Input: part model. Units: mm. Frame: model coordinates. Face numbers are marked on the shaded views. Coordinates: 2 decimals unless noted, no trailing zeros.
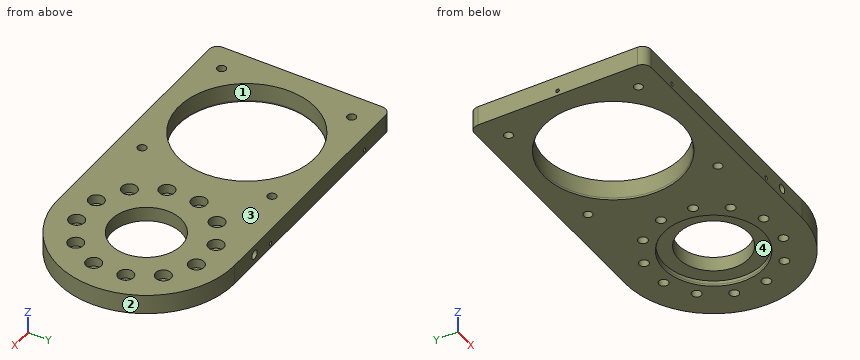
from build123d import *

# Parameters (mm, degrees)
BOSS_EXTRUDE1_DEPTH                                  = 23
FILLET1_R                                            = 10
HOLE_SIZE_PER_SOCKET_HEAD_CAP_SCREW_TYPE_D           = 11
HOLE_SIZE_PER_SOCKET_HEAD_CAP_SCREW_TYPE_CBORE_D     = 18
HOLE_SIZE_PER_SOCKET_HEAD_CAP_SCREW_TYPE_CBORE_DEPTH = 11
CIRPATTERN1_COUNT                                    = 12
SKETCH8_R                                            = 80
CUT_EXTRUDE1_DEPTH                                   = 23
SKETCH13_R                                           = 41
CUT_EXTRUDE3_DEPTH                                   = 23
SKETCH14_R                                           = 57.5
CUT_EXTRUDE4_DEPTH                                   = 6
M12_TAPPED_HOLE2_D                                   = 10.2
M5_TAPPED_HOLE1_AT_2_COUNT                           = 2
M5_TAPPED_HOLE1_AT_2_PITCH                           = 180
CHAMFER3_SIZE                                        = 2
CHAMFER3_SIZE2                                       = 0.727940469
CHAMFER4_SIZE                                        = 2
CHAMFER4_SIZE2                                       = 0.727940469
M5_TAPPED_HOLE3_D                                    = 4.2
M5_TAPPED_HOLE3_DEPTH                                = 12.4
M5_TAPPED_HOLE3_TIP                                  = 1.2618073


with BuildPart() as part:
    # Sketch1 → Boss-Extrude1 (new body)
    with BuildSketch(Plane.XY):
        with BuildLine():
            Line((0, 0), (298.3, 0))
            ThreePointArc((298.3, 0), (401.6, 103.3), (298.3, 206.6))
            Line((298.3, 206.6), (0, 206.6))
            Line((0, 206.6), (0, 0))
        make_face()
    extrude(amount=BOSS_EXTRUDE1_DEPTH)

    # Fillet1
    fillet1_edges = [part.edges().sort_by_distance(p)[0] for p in [
        (0, 206.6, 11.5),
        (0, 0, 11.5),
    ]]
    fillet(fillet1_edges, radius=FILLET1_R)

    # Hole Size per Socket Head Cap Screw Type3 (through all)
    with Locations(Plane.XY.offset(23)):
        with Locations((368.329622406, 84.53561923)):
            hole_size_per_socket_head_cap_screw_type = CounterBoreHole(HOLE_SIZE_PER_SOCKET_HEAD_CAP_SCREW_TYPE_D / 2, HOLE_SIZE_PER_SOCKET_HEAD_CAP_SCREW_TYPE_CBORE_D / 2, HOLE_SIZE_PER_SOCKET_HEAD_CAP_SCREW_TYPE_CBORE_DEPTH)

    # CirPattern1: Hole Size per Socket Head Cap Screw Type3 ×12 about axis
    cirpattern1_axis = Axis((298.3, 103.3, 0), (0, 0, 1))
    for i in range(1, CIRPATTERN1_COUNT):
        add(hole_size_per_socket_head_cap_screw_type.rotate(cirpattern1_axis, i * 360 / CIRPATTERN1_COUNT), mode=Mode.SUBTRACT)

    # Sketch8 → Cut-Extrude1 (cut)
    with BuildSketch(Plane.XY.offset(23)):
        with Locations((106.3, 103.3)):
            Circle(SKETCH8_R)
    extrude(amount=-CUT_EXTRUDE1_DEPTH, mode=Mode.SUBTRACT)

    # Sketch13 → Cut-Extrude3 (cut)
    with BuildSketch(Plane(origin=(0, 0, 0), x_dir=(-1, 0, 0), z_dir=(0, 0, -1))):
        with Locations((-298.3, 103.3)):
            Circle(SKETCH13_R)
    extrude(amount=-CUT_EXTRUDE3_DEPTH, mode=Mode.SUBTRACT)

    # Sketch14 → Cut-Extrude4 (cut)
    with BuildSketch(Plane(origin=(0, 0, 0), x_dir=(-1, 0, 0), z_dir=(0, 0, -1))):
        with Locations((-298.3, 103.3)):
            Circle(SKETCH14_R)
    extrude(amount=-CUT_EXTRUDE4_DEPTH, mode=Mode.SUBTRACT)

    # M12 Tapped Hole2 (through all)
    with Locations(Plane(origin=(0, 0, 0), x_dir=(-1, 0, 0), z_dir=(0, 0, -1))):
        with Locations((-30.286021022, 27.286021022), (-182.313978978, 27.286021022), (-30.286021022, 179.313978978), (-182.313978978, 179.313978978), (-106.3, 103.3)):
            Hole(M12_TAPPED_HOLE2_D / 2)

    # Sketch18 → M5 Tapped Hole1 (revolve, cut)
    with BuildSketch(Plane(origin=(50, 206.6, 5.5), x_dir=(0, 0, 1), z_dir=(1, 0, 0))):
        Polygon((0, 0), (0, 13.6618073), (2.1, 12.4), (2.1, 0), align=None)
    m5_tapped_hole1 = revolve(axis=Axis((50, 212.95, 5.5), (0, -1, 0)), mode=Mode.SUBTRACT)

    # M5 Tapped Hole1 at 2: M5 Tapped Hole1 ×2
    with Locations(*[(i * M5_TAPPED_HOLE1_AT_2_PITCH, 0, 0) for i in range(1, M5_TAPPED_HOLE1_AT_2_COUNT)]):
        add(m5_tapped_hole1, mode=Mode.SUBTRACT)

    # Mirror1: M5 Tapped Hole1 across plane
    add(m5_tapped_hole1.mirror(Plane.ZX.offset(103.3)), mode=Mode.SUBTRACT)

    # Mirror1 copy 1 sketch → Mirror1 copy 1 (revolve, cut)
    with BuildSketch(Plane(origin=(230, 0, 5.5), x_dir=(0, 0, 1), z_dir=(1, 0, 0))):
        Polygon((0, 0), (0, -13.6618073), (2.1, -12.4), (2.1, 0), align=None)
    revolve(axis=Axis((230, -6.35, 5.5), (0, -1, 0)), mode=Mode.SUBTRACT)

    # Chamfer3
    chamfer3_edges = [part.edges().sort_by_distance(p)[0] for p in [
        (26.3, 103.3, 0),
    ]]
    chamfer3_side = [part.faces().sort_by_distance(p)[0] for p in [
        (26.3, 103.3, 11.5),
    ]]
    chamfer(chamfer3_edges, length=CHAMFER3_SIZE, length2=CHAMFER3_SIZE2, reference=chamfer3_side[0])

    # Chamfer4
    chamfer4_edges = [part.edges().sort_by_distance(p)[0] for p in [
        (355.8, 103.3, 0),
    ]]
    chamfer4_side = [part.faces().sort_by_distance(p)[0] for p in [
        (355.8, 103.3, 3),
    ]]
    chamfer(chamfer4_edges, length=CHAMFER4_SIZE, length2=CHAMFER4_SIZE2, reference=chamfer4_side[0])

    # Sketch44 → M12 Tapped Hole3 (revolve, cut)
    with BuildSketch(Plane(origin=(260.3, 0, 11.5), x_dir=(0, 0, -1), z_dir=(1, 0, 0))):
        Polygon((0, 0), (0, 30.314389157), (5.1, 27.25), (5.1, 0), align=None)
    m12_tapped_hole3 = revolve(axis=Axis((260.3, -6.35, 11.5), (0, 1, 0)), mode=Mode.SUBTRACT)

    # Mirror5: M12 Tapped Hole3 across plane
    add(m12_tapped_hole3.mirror(Plane(origin=(0, 103.3, 0), x_dir=(0, 0, 1), z_dir=(0, -1, 0))), mode=Mode.SUBTRACT)

    # M5 Tapped Hole3
    with Locations(Plane.ZY):
        with Locations((5.5, 103.3)):
            Hole(M5_TAPPED_HOLE3_D / 2, depth=M5_TAPPED_HOLE3_DEPTH)
            with Locations((0, 0, -(M5_TAPPED_HOLE3_DEPTH + M5_TAPPED_HOLE3_TIP / 2))):  # 118° drill point
                Cone(0, M5_TAPPED_HOLE3_D / 2, M5_TAPPED_HOLE3_TIP, mode=Mode.SUBTRACT)


solid = part.part
Item 1: Material intervals for line 1 (X direction, y = 110, z = 15.5); line 2 (X direction, y = 87.5, z = 11.5); line 3 (X direction, y = 23, z = 8.5), sorted ascending.
Item 2: Pin query (flat end, axial travel): pin 1 Ø3 at (y, z) = (37.5, 9.5) entering from +X; pin 2 Ø1 at (y, z) = (76, 18.5) entering from +X; pin 3 Ø9 at (x, z) = (260.3, 11.5) entering from +Y. Return the tip coordinate at first contact, or that it passes through.
Item 3: Pull-direction query (Y, two-part tool) for the marked faces 1, 2, 3 and 4; classes: released by +Y, released by -Y, zero draft, split by the parting line, or undercut.
The answers:
1. line 1: x = 0 to 26.58, 186.02 to 257.85, 338.75 to 401.38
1. line 2: x = 0 to 27.88, 184.72 to 223.64, 232.9 to 260.47, 336.13 to 363.7, 372.96 to 400.38
1. line 3: x = 0 to 27.52, 33.05 to 179.55, 185.08 to 256.18, 264.42 to 363.28
2. pin 1: stops at x = 379.15
2. pin 2: stops at x = 398.06
2. pin 3: stops at y = 178.99
3. face 1: undercut
3. face 2: split by the parting line
3. face 3: zero draft
3. face 4: undercut
